Build history of the part. All positions in model axes, mm. A direction names the side the tool comes from. Give positions to 0.01 mm unless a question says otherwise; leave off trailing zeros. Loops run counter-clockwise (first coordinate to the right, second up) from the corner with the lowest first, then second, coordinate; pieces in that order, holes last. Notation, with made-up numbers: M -35.75,79 L -15.75,79 A26 ccw -15.75,112 Z; hole C 65,35.5 d9. An arc over 180 degrees is marked long. Put each result on its own line as item: value.
```python
from build123d import *

# Parameters (mm, degrees)
SKETCH_1_W              = 70
SKETCH_1_H              = 55
EXTRUDE_1_DEPTH         = 10
SKETCH_2_W              = 10
SKETCH_2_H              = 45
CUT_EXTRUDE_1_DEPTH     = 46.620718977
SKETCH_3_R              = 17
CUT_EXTRUDE_2_DEPTH     = 46.620718977
HOLE_WIZARD_M4_2_D      = 3.3
HOLE_WIZARD_5_5_5_5_1_D = 5.5
CHAMFER_1_SIZE          = 5
SKETCH_12_W             = 24
SKETCH_12_H             = 9
CUT_EXTRUDE_3_DEPTH     = 46.620718977
CHAMFER_2_SIZE          = 0.5


with BuildPart() as part:
    # 草图1 → 凸台-拉伸1 (new body)
    with BuildSketch(Plane.XY):
        Rectangle(SKETCH_1_W, SKETCH_1_H)
    extrude(amount=EXTRUDE_1_DEPTH)

    # 草图2 → 切除-拉伸1 (cut, through all)
    with BuildSketch(Plane.XY.offset(10)):
        with Locations((-30, -5)):
            Rectangle(SKETCH_2_W, SKETCH_2_H)
        with Locations((30, -5)):
            Rectangle(SKETCH_2_W, SKETCH_2_H)
    extrude(amount=-CUT_EXTRUDE_1_DEPTH, mode=Mode.SUBTRACT)

    # 草图3 → 切除-拉伸2 (cut, through all)
    with BuildSketch(Plane(origin=(0, 0, 0), x_dir=(-1, 0, 0), z_dir=(0, 0, -1))):
        with Locations((0, -6.5)):
            Circle(SKETCH_3_R)
    extrude(amount=-CUT_EXTRUDE_2_DEPTH, mode=Mode.SUBTRACT)

    # M4 螺纹孔2 (through all)
    with Locations(Plane.XY.offset(10)):
        with Locations((14.85, -21.35), (-14.85, -21.35), (-14.85, 8.35), (14.85, 8.35)):
            Hole(HOLE_WIZARD_M4_2_D / 2)

    # Ø5.5 (5.5) 直径孔1 (through all)
    with Locations(Plane(origin=(0, 17.5, 0), x_dir=(-1, 0, 0), z_dir=(0, -1, 0))):
        with Locations((-30, -5), (30, -5)):
            Hole(HOLE_WIZARD_5_5_5_5_1_D / 2)

    # 倒角1
    chamfer_1_edges = [part.edges().sort_by_distance(p)[0] for p in [
        (-25, -27.5, 5),
        (25, -27.5, 5),
    ]]
    chamfer(chamfer_1_edges, length=CHAMFER_1_SIZE)

    # 草图12 → 切除-拉伸3 (cut, through all)
    with BuildSketch(Plane.XY.offset(10)):
        with Locations((0, 23)):
            Rectangle(SKETCH_12_W, SKETCH_12_H)
    extrude(amount=-CUT_EXTRUDE_3_DEPTH, mode=Mode.SUBTRACT)

    # 倒角2
    chamfer_2_edges = [part.edges().sort_by_distance(p)[0] for p in [
        (-35, 22.5, 10),
        (0, 18.5, 10),
        (12, 23, 10),
        (-30, 17.5, 0),
        (-35, 17.5, 5),
        (-30, 17.5, 10),
        (35, 22.5, 0),
        (35, 22.5, 10),
        (25, -2.5, 0),
        (30, 17.5, 0),
        (35, 17.5, 5),
        (30, 17.5, 10),
        (25, -2.5, 10),
        (-35, 22.5, 0),
        (23.5, 27.5, 0),
        (23.5, 27.5, 10),
        (-35, 27.5, 5),
        (35, 27.5, 5),
        (-25, -2.5, 10),
        (-25, -2.5, 0),
        (0, -27.5, 10),
        (22.5, -25, 10),
        (-22.5, -25, 10),
        (0, -27.5, 0),
        (22.5, -25, 0),
        (-22.5, -25, 0),
        (-23.5, 27.5, 0),
        (-23.5, 27.5, 10),
        (-12, 23, 0),
        (12, 23, 0),
        (0, 18.5, 0),
        (-12, 23, 10),
    ]]
    chamfer(chamfer_2_edges, length=CHAMFER_2_SIZE)


solid = part.part
```
Q1. Slice it at C-C (z = 8.75). List the corners of the cut face in (x, y).
Here are the results:
outline: M -35,18 L -34.5,17.5 L -25,17.5 L -25,-22.5 L -20,-27.5 L 20,-27.5 L 25,-22.5 L 25,17.5 L 34.5,17.5 L 35,18 L 35,27 L 34.5,27.5 L 12,27.5 L 12,18.5 L -12,18.5 L -12,27.5 L -34.5,27.5 L -35,27 Z; hole C 0,-6.5 d34; hole C -14.85,-21.35 d3.3; hole C -14.85,8.35 d3.3; hole C 14.85,-21.35 d3.3; hole C 14.85,8.35 d3.3
Q2. Probe line 1 (Y direction, x = 0, z = 6.5); line 2 (Y direction, x = -13.5, z = 8.75); line 3 (Y direction, x = 15, z = 9.75). List the from-to ranges inside material, lowest first. Write a range as from..to.
Here are the results:
line 1: -27.5..-23.5, 10.5..18.5
line 2: -27.5..-22.3, -20.4..-16.83, 3.83..7.4, 9.3..27.5
line 3: -27.25..-22.99, -19.71..-14.5, 1.5..6.71, 9.99..27.25
Q3. Slice it at D-D (x = 0). List the corners of the cut face in (y, z), and give its area (4 significant figures).
Here are the results:
outline: M -27.5,0.5 L -27,0 L -23.5,0 L -23.5,10 L -27,10 L -27.5,9.5 Z; M 10.5,0 L 18,0 L 18.5,0.5 L 18.5,9.5 L 18,10 L 10.5,10 Z
area: 119.5 mm²
Q4. Drop flat-ended pins along their axis: pin 1 Ø6 at (y, z) = (-17.5, 1.5) entering from -X; pin 2 Ø2.5 at (y, z) = (4, 7) entering from +X; pin 3 Ø4.5 at (x, z) = (-28.5, 5) entering from -Y. Give the stop position or say it passes through.
Here are the results:
pin 1: x = -25
pin 2: x = 25
pin 3: y = 17.5
Q5. Slice it at A-A (z = 5). State how many separate pieces and enclosed holes the cut face has, and give its area (3 significant figures).
Here are the results:
separate pieces: 3
enclosed holes: 5
area: 1,660 mm²
Q6. Mould opens along X. For faces 1 (the flat face through (23, 27.5, 5)), 2 (the cylindrical face through (13.491, -16.844, 4.93)), 3 (the flat face through (25, -3, 5)), 4 (the flat face through (-12, 23, 5)) say: pulls with the +X half, pulls with the -X half, needs draft (parallel to the pull), parting line crosses it, or undercut.
Here are the results:
face 1: needs draft
face 2: undercut
face 3: pulls with the +X half
face 4: undercut
Q7. Tool access for faces 5 (the flat face through (0, 18.5, 5)), 6 (the flat face through (-27.7, 17.5, 7.1)), 7 (the flat face through (27.6, 17.5, 3.1)), 8 (the cylindrical face through (14.089, -22.814, 4.93)): list every direction of +Z, -Z, +X, -X, +Y, -Y with a clear straight run to the whole face (end or side of a thin tool).
Here are the results:
face 5: +Z, -Z, +Y
face 6: +Z, -Z, -X, -Y
face 7: +Z, -Z, +X, -Y
face 8: +Z, -Z
Q8. Slice it at B-B (y = -6.5). List the corners of the cut face in (x, z), and give its area (4 significant figures).
Here are the results:
outline: M -25,0.5 L -24.5,0 L -17,0 L -17,10 L -24.5,10 L -25,9.5 Z; M 17,0 L 24.5,0 L 25,0.5 L 25,9.5 L 24.5,10 L 17,10 Z
area: 159.5 mm²
